Model file for the job. Use its own axes, mm. A direction names the side the tool comes from. Round coordinates to 2 decimals unless told otherwise and drop trailing zeros. Loops run counter-clockwise (first coordinate to the right, second up) from the corner with the lowest first, then second, coordinate; pieces in that order, holes last. Notation, with made-up numbers: M -39.75,-29.5 L -34.75,-29.5 A30 cw -34.75,1.5 Z; hole C 86.25,42.25 d1. An arc over 180 degrees is marked long. Use a Markdown table: item, result. Add a question column.
Item 1: Pin check, flat tips, straight feed: P1, Ø12, axis at x = 15, y = 55, coming from the +Z side; P2, Ø1.5, axis at x = -21.5, y = 66.5, coming from the -Z side; P3, Ø10, axis at x = 0, z = -32.5, coming from the +Y side; P4, Ø2, axis at x = 6, y = 29.5, coming from the +Z side. Stop position of each tip, or through.
Item 2: Saw through at C-C on y = 36.5. Write the cut outline in (x, z), then the cut area to 3 significant figures.
Item 3: Wall check: L1, parallel to X at y = 37.5, z = 0; L2, parallel to X at y = 53.5, z = -9; L3, parallel to Z at x = 20, y = 58.5. Give the ranges that are in metal, low to high. Write a range as from..to.
Item 4: Tool access for faces 1 (the cylindrical face through (7.509, 71.464, 23.846)), 2 (the cylindrical face through (-36.303, 7.199, -6.991)), 3 (the flat face through (-17, 58.4, -17)): list every direction of +Z, -Z, +X, -X, +Y, -Y with a clear straight run to the whole face (end or side of a thin tool).
Item 5: Saw through at A-A on y = 83. Write the cut outline in (x, z), then the cut area to 3 significant figures.
Item 6: Two-plate mould, pull along Z, no slides. Class faces 4 (the flat face through (-18, 14.2, 18)), 5 (the cylindrical face through (-17.235, 5.275, 41.569)), 6 (the conical face through (5.77, 0.95, 13.91)): +Z half, -Z half, draft (parallel to the pull), parting line (faces both ways), or undercut.
Item 7: Saw through at B-B on z = 0. Give the number of separate pieces and of enclosed holes in the cut face, then the cut area to 3 significant figures.
```python
from build123d import *

# Parameters (mm, degrees)
FLANGE_SKETCH_R                = 45
FLANGE_90_DEPTH                = 14.2
NECK_SKETCH_R                  = 20
NECK_40_DEPTH                  = 44.2
HEAD_SKETCH_R                  = 25
HEAD_50_DEPTH                  = 30
BOLT_HOLE_1_SKETCH_R           = 6.25
BOLT_HOLE_1_12_5_DEPTH         = 30
BOLT_HOLE_2_SKETCH_R           = 6.25
BOLT_HOLE_2_12_5_DEPTH         = 30
BOLT_HOLE_3_SKETCH_R           = 6.25
BOLT_HOLE_3_12_5_DEPTH         = 30
BOLT_HOLE_4_SKETCH_R           = 6.25
BOLT_HOLE_4_12_5_DEPTH         = 30
COUNTERBORE_SKETCH_R           = 19
COUNTERBORE_38_DEPTH           = 12
BORE_STEP_SKETCH_R             = 19
BORE_STEP_DEPTH_12_DEPTH       = 12
INNER_BORE_SKETCH_R            = 15
INNER_BORE_30_DEPTH            = 6
NECK_BORE_SKETCH_R             = 15
NECK_BORE_DEPTH                = 44.2
BOTTOM_RECESS_SKETCH_R         = 15
BOTTOM_RECESS_30_DRAFTED_DEPTH = 3.5
BOTTOM_RECESS_30_DRAFTED_DRAFT = 3.5
THROUGH_BORE_SKETCH_R          = 15
THROUGH_BORE_DEPTH             = 80.5
FLANGE_NECK_FILLET_R3_5_R      = 3.5
HEAD_EDGE_FILLET_R3_5_R        = 3.5
NECK_HEAD_FILLET_R3_5_R        = 3.5
FLANGE_EDGE_FILLET_R3_5_R      = 3.5


with BuildPart() as part:
    # Flange Sketch → Flange Ø90 (new body)
    with BuildSketch(Plane(origin=(0, 0, 0), x_dir=(1, 0, 0), z_dir=(0, 1, 0))):
        with Locations(Location((0, 0, 0), (0, 0, 270))):
            Circle(FLANGE_SKETCH_R)
    extrude(amount=FLANGE_90_DEPTH)

    # Neck Sketch → Neck Ø40 (add)
    with BuildSketch(Plane(origin=(0, 14.2, 0), x_dir=(1, 0, 0), z_dir=(0, 1, 0))):
        with Locations(Location((0, 0, 0), (0, 0, 270))):
            Circle(NECK_SKETCH_R)
    extrude(amount=NECK_40_DEPTH)

    # Head Sketch → Head Ø50 (add)
    with BuildSketch(Plane(origin=(0, 58.4, 0), x_dir=(1, 0, 0), z_dir=(0, 1, 0))):
        with Locations(Location((0, 0, 0), (0, 0, 270))):
            Circle(HEAD_SKETCH_R)
    extrude(amount=HEAD_50_DEPTH)

    # Bolt Hole 1 Sketch → Bolt Hole 1 Ø12.5 (cut)
    with BuildSketch(Plane(origin=(0, 14.2, 0), x_dir=(1, 0, 0), z_dir=(0, 1, 0))):
        with Locations(Location((0, 32.5, 0), (0, 0, 270))):
            Circle(BOLT_HOLE_1_SKETCH_R)
    extrude(amount=-BOLT_HOLE_1_12_5_DEPTH, mode=Mode.SUBTRACT)

    # Bolt Hole 2 Sketch → Bolt Hole 2 Ø12.5 (cut)
    with BuildSketch(Plane(origin=(0, 14.2, 0), x_dir=(1, 0, 0), z_dir=(0, 1, 0))):
        with Locations(Location((32.5, 0, 0), (0, 0, 270))):
            Circle(BOLT_HOLE_2_SKETCH_R)
    extrude(amount=-BOLT_HOLE_2_12_5_DEPTH, mode=Mode.SUBTRACT)

    # Bolt Hole 3 Sketch → Bolt Hole 3 Ø12.5 (cut)
    with BuildSketch(Plane(origin=(0, 14.2, 0), x_dir=(1, 0, 0), z_dir=(0, 1, 0))):
        with Locations(Location((-32.5, 2.030932752, 0), (0, 0, 270))):
            Circle(BOLT_HOLE_3_SKETCH_R)
    extrude(amount=-BOLT_HOLE_3_12_5_DEPTH, mode=Mode.SUBTRACT)

    # Bolt Hole 4 Sketch → Bolt Hole 4 Ø12.5 (cut)
    with BuildSketch(Plane(origin=(0, 14.2, 0), x_dir=(1, 0, 0), z_dir=(0, 1, 0))):
        with Locations(Location((-1.69244396, -32.5, 0), (0, 0, 270))):
            Circle(BOLT_HOLE_4_SKETCH_R)
    extrude(amount=-BOLT_HOLE_4_12_5_DEPTH, mode=Mode.SUBTRACT)

    # Counterbore Sketch → Counterbore Ø38 (cut)
    with BuildSketch(Plane(origin=(0, 88.4, 0), x_dir=(1, 0, 0), z_dir=(0, 1, 0))):
        with Locations(Location((0, 0, 0), (0, 0, 270))):
            Circle(COUNTERBORE_SKETCH_R)
    extrude(amount=-COUNTERBORE_38_DEPTH, mode=Mode.SUBTRACT)

    # Bore Step Sketch → Bore Step Depth 12 (cut)
    with BuildSketch(Plane(origin=(0, 76.4, 0), x_dir=(1, 0, 0), z_dir=(0, 1, 0))):
        with Locations(Location((0, 0, 0), (0, 0, 270))):
            Circle(BORE_STEP_SKETCH_R)
    extrude(amount=-BORE_STEP_DEPTH_12_DEPTH, mode=Mode.SUBTRACT)

    # Inner Bore Sketch → Inner Bore Ø30 (cut)
    with BuildSketch(Plane(origin=(0, 64.4, 0), x_dir=(1, 0, 0), z_dir=(0, 1, 0))):
        with Locations(Location((0, 0, 0), (0, 0, 270))):
            Circle(INNER_BORE_SKETCH_R)
    extrude(amount=-INNER_BORE_30_DEPTH, mode=Mode.SUBTRACT)

    # Neck Bore Sketch → Neck Bore (cut)
    with BuildSketch(Plane(origin=(0, 58.4, 0), x_dir=(1, 0, 0), z_dir=(0, 1, 0))):
        with Locations(Location((0, 0, 0), (0, 0, 270))):
            Circle(NECK_BORE_SKETCH_R)
    extrude(amount=-NECK_BORE_DEPTH, mode=Mode.SUBTRACT)


with BuildPart() as bottom_recess_30_drafted_tool:
    # Bottom Recess Sketch → Bottom Recess Ø30 Drafted (with draft: the straight prism first)
    with BuildSketch(Plane.XZ):
        with Locations(Location((0, 0, 0), (0, 0, 90))):
            Circle(BOTTOM_RECESS_SKETCH_R)
    extrude(amount=-BOTTOM_RECESS_30_DRAFTED_DEPTH)
    # Bottom Recess Ø30 Drafted: the draft: its side faces are tilted about the plane it starts from
    bottom_recess_30_drafted_sides = [bottom_recess_30_drafted_tool.faces().sort_by_distance(p)[0] for p in [
        (0, 1.75, -15),
    ]]
    draft(bottom_recess_30_drafted_sides, Plane.XZ, BOTTOM_RECESS_30_DRAFTED_DRAFT)


with BuildPart() as part_1:
    add(part.part)

    # Bottom Recess Ø30 Drafted: cut by bottom_recess_30_drafted_tool
    add(bottom_recess_30_drafted_tool.part, mode=Mode.SUBTRACT)

    # Through Bore Sketch → Through Bore (cut)
    with BuildSketch(Plane(origin=(0, 14.2, 0), x_dir=(1, 0, 0), z_dir=(0, 1, 0))):
        with Locations(Location((0, 0, 0), (0, 0, 270))):
            Circle(THROUGH_BORE_SKETCH_R)
    extrude(amount=-THROUGH_BORE_DEPTH, mode=Mode.SUBTRACT)

    # Flange-Neck Fillet R3.5
    flange_neck_fillet_r3_5_edges = [part_1.edges().sort_by_distance(p)[0] for p in [
        (0, 14.2, -20),
    ]]
    fillet(flange_neck_fillet_r3_5_edges, radius=FLANGE_NECK_FILLET_R3_5_R)

    # Head Edge Fillet R3.5
    head_edge_fillet_r3_5_edges = [part_1.edges().sort_by_distance(p)[0] for p in [
        (0, 88.4, -25),
    ]]
    fillet(head_edge_fillet_r3_5_edges, radius=HEAD_EDGE_FILLET_R3_5_R)

    # Neck-Head Fillet R3.5
    neck_head_fillet_r3_5_edges = [part_1.edges().sort_by_distance(p)[0] for p in [
        (0, 58.4, -20),
    ]]
    fillet(neck_head_fillet_r3_5_edges, radius=NECK_HEAD_FILLET_R3_5_R)

    # Flange Edge Fillet R3.5
    flange_edge_fillet_r3_5_edges = [part_1.edges().sort_by_distance(p)[0] for p in [
        (0, 14.2, -45),
    ]]
    fillet(flange_edge_fillet_r3_5_edges, radius=FLANGE_EDGE_FILLET_R3_5_R)


solid = part_1.part
```
Entries:
| question | item | result |
|---|---|---|
| 1 | P1 | z = 22.89 |
| 1 | P2 | z = -13.94 |
| 1 | P3 | through |
| 1 | P4 | z = 19.36 |
| 2 | outline | C 0,0 d40; hole C 0,0 d30 |
| 2 | area | 550 mm2 |
| 3 | L1 | -20..-15, 15..20 |
| 3 | L2 | -17.86..-12, 12..17.86 |
| 3 | L3 | -15..15 |
| 4 | face 1 | +Y |
| 4 | face 2 | +Y, -Y |
| 4 | face 3 | none |
| 5 | outline | C 0,0 d50; hole C 0,0 d38 |
| 5 | area | 829 mm2 |
| 6 | face 4 | draft |
| 6 | face 5 | parting line |
| 6 | face 6 | undercut |
| 7 | separate pieces | 4 |
| 7 | enclosed holes | 0 |
| 7 | area | 1,360 mm2 |
